Here's the drawing with two shaded views (mm, measured from the low corner). I have some questions. Give positions to 0.01 mm unless a question says otherwise; leave off trailing zeros. Loops run counter-clockwise (first coordinate to the right, second up) from the corner with the lowest first, then second, coordinate; pieces in that order, holes last. Notation, with made-up numbers: M 29.5,-27.75 L 60.5,-27.75 A30 ccw 60.5,11.25 Z; hole C 68,79 d8. An arc over 180 degrees is marked long. Use CSV: the item, a comma, the result in double quotes.
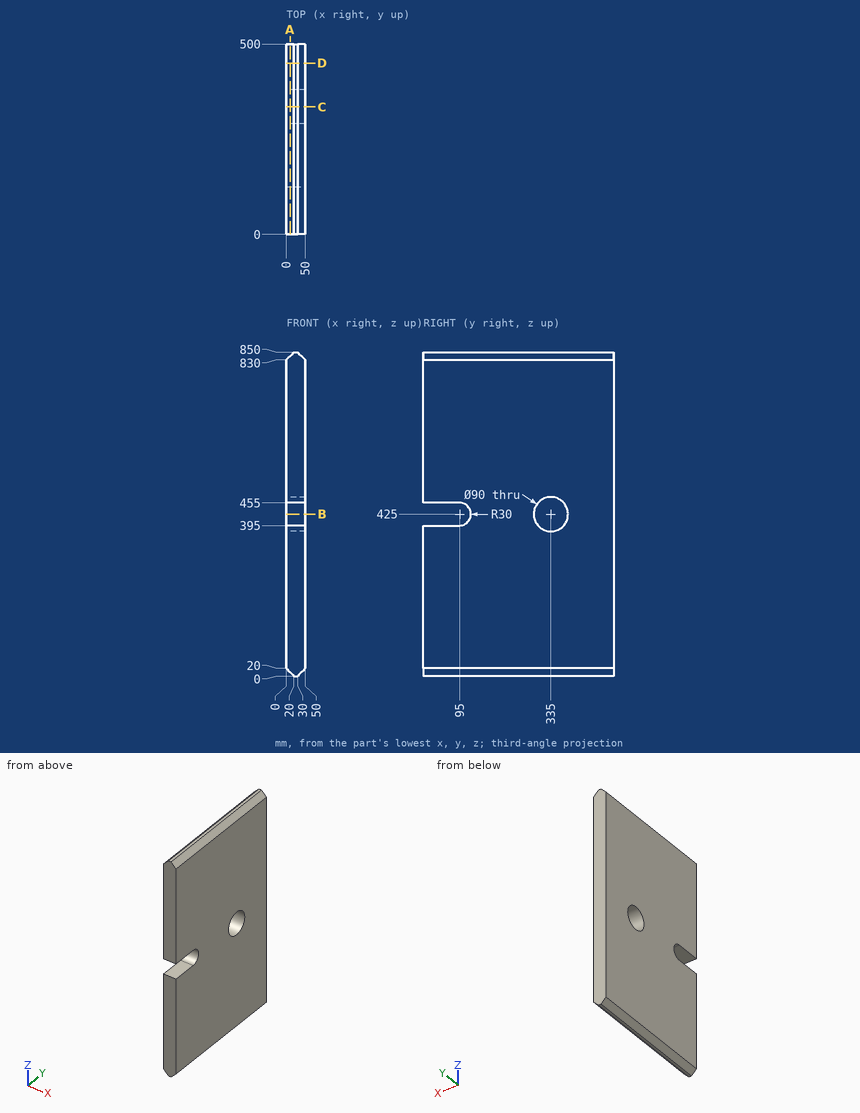
1. I want a section at D-D, the plane y = 450. List the corners of the cut face in (x, z) for me.
Outcome:
outline,"M 0,20 L 20,0 L 30,0 L 50,20 L 50,830 L 30,850 L 20,850 L 0,830 Z"
2. Please list where these lines run through material, in increasing order: line 1 (Y direction, x = 39, z = 425); line 2 (Z direction, x = 25, y = 97); line 3 (Z direction, x = 45, y = 304).
Outcome:
line 1,"125 to 290, 380 to 500"
line 2,"0 to 395.07, 454.93 to 850"
line 3,"15 to 392.38, 457.62 to 835"
3. I'm going to push flat-ended pins straight in: pin 1 Ø10 at (x, y) = (39.5, 136) entering from -Z; pin 2 Ø8 at (x, y) = (5.5, 346) entering from +Z; pin 3 Ø6 at (x, y) = (35.5, 365.5) entering from +Z. Where does each tip first touch, or does it pass through?
Outcome:
pin 1,"z = 4.5"
pin 2,"z = 839.5"
pin 3,"z = 847.5"
4. I want a section at A-A, the plane x = 10. List the corners of the cut face in (y, z) for me.
Outcome:
outline,"M 0,10 L 500,10 L 500,840 L 0,840 L 0,455 L 95,455 A30 cw 95,395 L 0,395 Z; hole C 335,425 d90"
5. I want a section at B-B, the plane z = 425. List the corners of the cut face in (x, y) for me, then the cut area to 4 significant figures.
Outcome:
outline,"M 0,125 L 50,125 L 50,290 L 0,290 Z; M 0,380 L 50,380 L 50,500 L 0,500 Z"
area,"14,250 mm2"
6. I want a section at C-C, the plane y = 335. List the corners of the cut face in (x, z) for me.
Outcome:
outline,"M 0,20 L 20,0 L 30,0 L 50,20 L 50,380 L 0,380 Z; M 0,470 L 50,470 L 50,830 L 30,850 L 20,850 L 0,830 Z"
